The model under review builds one solid part; all positions refer to its coordinate system, in mm. Round coordinates to 2 decimals unless told otherwise and drop trailing zeros. Write each loop counter-clockwise with the first axis right and the second up, starting at its lowest first coordinate (ties: lowest second). Pieces come first, ordered by that corner, then holes. Notation, with made-up numbers: (7.5, 6) - (61.5, 6) arc R13 ccw to (61.5, 23) - close; hole circle Ø6 at (-18.75, 0.5). An arc over 180 degrees is marked (long way). Use one line per item in the form item = value.
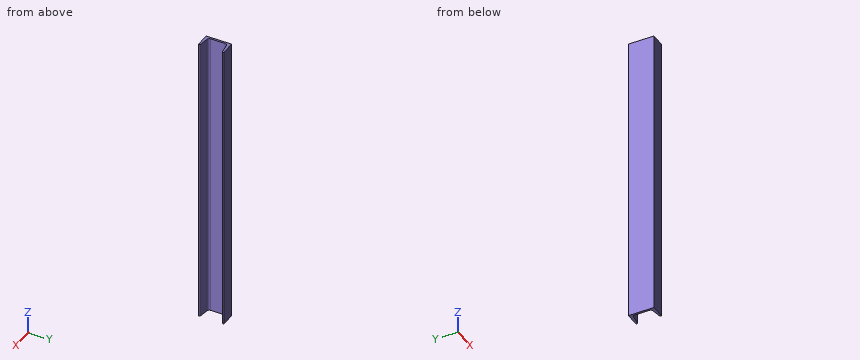
from build123d import *

# Parameters (mm, degrees)
BOSS_EXTRUDE1_DEPTH = 920


with BuildPart() as part:
    # Sketch1 → Boss-Extrude1 (new body)
    with BuildSketch(Plane.XY):
        with BuildLine():
            Line((0, 0), (-45, 0))
            Line((-45, 0), (-45, -80))
            Line((-45, -80), (0, -80))
            Line((0, -80), (0, -78.639315732))
            ThreePointArc((0, -78.639315732), (-0.981161679, -76.015079616), (-3.443307596, -74.678243457))
            Line((-3.443307596, -74.678243457), (-32.113384808, -70.648926875))
            ThreePointArc((-32.113384808, -70.648926875), (-37.037676642, -67.975254557), (-39, -62.726782325))
            Line((-39, -62.726782325), (-39, -17.273217675))
            ThreePointArc((-39, -17.273217675), (-37.037676642, -12.024745443), (-32.113384808, -9.351073125))
            Line((-32.113384808, -9.351073125), (-3.443307596, -5.321756543))
            ThreePointArc((-3.443307596, -5.321756543), (-0.981161679, -3.984920384), (0, -1.360684268))
            Line((0, -1.360684268), (0, 0))
        make_face()
    extrude(amount=BOSS_EXTRUDE1_DEPTH)


solid = part.part
(1) To check wall thickness, follow L1, parallel to X at y = -40, z = 493.5; L2, parallel to Y at x = -8, z = 751; L3, parallel to Y at x = -33.5, z = 866.5. State the ranges of each line that lie inside material, in increasing order.
Geometry results:
L1 = -45 to -39
L2 = -80 to -74.04, -5.96 to 0
L3 = -80 to -70.33, -9.67 to 0
(2) Insertion check: P1, Ø8, axis at x = -33.5, z = 294.5, coming from the +Y side. The pin has a flat end and moves straight along its axis. Give the tip position at first contact, or say it passes through.
Geometry results:
P1 = 0
(3) Add section B-B on z = 93. Write out the cut boundary in (x, y), then the cut area to 3 significant figures.
Geometry results:
outline = (-45, -80) - (0, -80) - (0, -78.64) arc R4 ccw to (-3.44, -74.68) - (-32.11, -70.65) arc R8 cw to (-39, -62.73) - (-39, -17.27) arc R8 cw to (-32.11, -9.35) - (-3.44, -5.32) arc R4 ccw to (0, -1.36) - (0, 0) - (-45, 0) - close
area = 1,090 mm2
(4) Add section C-C on y = -32.5. Write out the cut boundary in (x, z), then the cut area to 3 significant figures.
Geometry results:
outline = (-45, 0) - (-39, 0) - (-39, 920) - (-45, 920) - close
area = 5,520 mm2
(5) Add section A-A on x = -24. Write out the cut boundary in (y, z).
Geometry results:
outline = (-80, 0) - (-71.79, 0) - (-71.79, 920) - (-80, 920) - close; (-8.21, 0) - (0, 0) - (0, 920) - (-8.21, 920) - close
